```python
from build123d import *

# Parameters (mm, degrees)
LINK_PROFILE_SKETCH_R   = 7.5
LINK_PROFILE_SKETCH_R_2 = 20.85
LINK_BODY_15MM_DEPTH    = 15
BOLT_HOLE_SKETCH_R      = 5
BOLT_HOLE_10_DEPTH      = 159.633571478


with BuildPart() as part:
    # Link Profile Sketch → Link Body 15mm (new body)
    with BuildSketch(Plane.XY):
        with BuildLine():
            Line((100, 47), (92, 47))
            ThreePointArc((92, 47), (90.104459839, 21.32227727), (67.496938967, 9))
            Line((67.496938967, 9), (11.618950039, 9))
            ThreePointArc((11.618950039, 9), (6, 11.237900077), (0, 12))
            ThreePointArc((0, 12), (-12, 0), (0, -12))
            ThreePointArc((0, -12), (6, -11.237900077), (11.618950039, -9))
            Line((11.618950039, -9), (67.496938967, -9))
            ThreePointArc((67.496938967, -9), (90.104459839, -21.32227727), (92, -47))
            Line((92, -47), (100, -47))
            Line((100, -47), (108.73655718, -47))
            ThreePointArc((108.73655718, -47), (109.975380436, -32.246626192), (118.119137608, -19.882325124))
            ThreePointArc((118.119137608, -19.882325124), (126.899218543, 0.205040931), (117.813941305, 20.156227206))
            ThreePointArc((117.813941305, 20.156227206), (109.504751294, 32.334280207), (108, 47))
            Line((108, 47), (100, 47))
        make_face()
        Circle(LINK_PROFILE_SKETCH_R, mode=Mode.SUBTRACT)
        with Locations((100, 0)):
            Circle(LINK_PROFILE_SKETCH_R_2, mode=Mode.SUBTRACT)
        with BuildLine():
            Line((22.3, -5), (58.3, -5))
            ThreePointArc((58.3, -5), (63.3, 0), (58.3, 5))
            Line((58.3, 5), (22.3, 5))
            ThreePointArc((22.3, 5), (17.3, 0), (22.3, -5))
        make_face(mode=Mode.SUBTRACT)
    extrude(amount=LINK_BODY_15MM_DEPTH)

    # Bolt Hole Sketch → Bolt Hole Ø10 (cut, through all)
    with BuildSketch(Plane.XZ.offset(47)):
        with Locations(Location((100.36827859, 7.5, 0), (0, 0, 270))):
            Circle(BOLT_HOLE_SKETCH_R)
    extrude(amount=-BOLT_HOLE_10_DEPTH, mode=Mode.SUBTRACT)


solid = part.part
```
Read the model definition and answer for the solid it produces. Units are mm, in the model's axes. A direction names the side the tool comes from. Give positions to 0.01 mm unless a question says otherwise; leave off trailing zeros. Loops run counter-clockwise (first coordinate to the right, second up) from the corner with the lowest first, then second, coordinate; pieces in that order, holes last.
Item 1: The part is cut by section A-A (z = 8.5). Write down the section's boundary in (x, y).
Item 2: The part is cut by section B-B (y = 0). Write down the section's boundary in (x, z), and give its area (3 significant figures).
Item 3: For faces 4 (the flat face through (39, -9, 7)), 5 (the cylindrical face through (63.3, -0.1, 7.4)), 6 (the flat face through (40, 9, 7)), 7 (the flat face through (73, 0, 15)), determine the directions among +Z, -Z, +X, -X, +Y, -Y from which every point of the face is accessible in a straight line to the end or side of a thin tool.
Item 4: The part is cut by section C-C (x = 34.5). Write down the section's boundary in (y, z), and give its area (3 significant figures).
Item 5: Find the intervals of material crossed by line 1 along X through (y, z) = (-2, 3); line 2 along X through (y, z) = (-41.5, 9.25); line 3 along X through (y, z) = (29, 7.5), in increasing order.
Item 6: Each of these flat-tipped pins is pushed along its axis until it touches: pin 1 Ø6 at (x, z) = (66, 9.5) entering from +Y; pin 2 Ø5 at (y, z) = (11.5, 2.5) entering from -X; pin 3 Ø1.5 at (y, z) = (-35, 9) entering from -X. Where does it stop, or does it pass through?
Item 7: The mould has two halves that part along Y. Classify faces 1 (the flat face through (73, 0, 0)), 2 (the cylindrical face through (109.91, -32.44, 7.4)), 3 (the cylindrical face through (-12, 0, 7)): released by +Y, released by -Y, zero draft, split by the parting line, or undercut.
Item 8: The part is cut by section D-D (y = 34). Write down the section's boundary in (x, z), and give its area (3 significant figures).
Taken from the geometry:
1. outline: (0, -12) arc R24 ccw to (11.62, -9) - (67.5, -9) arc R26.9 cw to (92, -47) - (95.47, -47) - (95.47, -20.35) arc R20.85 cw to (95.47, 20.35) - (95.47, 47) - (92, 47) arc R26.9 cw to (67.5, 9) - (11.62, 9) arc R24 ccw to (0, 12) arc R12 ccw to start; (105.27, -47) - (108.74, -47) arc R30 cw to (118.12, -19.88) arc R26.9 ccw to (117.81, 20.16) arc R30 cw to (108, 47) - (105.27, 47) - (105.27, 20.17) arc R20.85 cw to (105.27, -20.17) - close; hole circle Ø15 at (0, 0); hole (22.3, -5) - (58.3, -5) arc R5 ccw to (58.3, 5) - (22.3, 5) arc R5 ccw to start
2. outline: (-12, 0) - (-7.5, 0) - (-7.5, 15) - (-12, 15) - close; (7.5, 0) - (17.3, 0) - (17.3, 15) - (7.5, 15) - close; (63.3, 0) - (79.15, 0) - (79.15, 15) - (63.3, 15) - close; (120.85, 0) - (126.9, 0) - (126.9, 15) - (120.85, 15) - close
2. area: 543 mm2
3. face 4: +Z, -Z, -Y
3. face 5: +Z, -Z
3. face 6: +Z, -Z, +Y
3. face 7: +Z, +X, -X, +Y, -Y
4. outline: (-9, 0) - (-5, 0) - (-5, 15) - (-9, 15) - close; (5, 0) - (9, 0) - (9, 15) - (5, 15) - close
4. area: 120 mm2
5. line 1: x = -11.83 to -7.23, 7.23 to 17.72, 62.88 to 79.25, 120.75 to 126.83
5. line 2: x = 93.81 to 95.68, 105.05 to 108.33
5. line 3: x = 93.5 to 95.37, 105.37 to 110.96
6. pin 1: stops at y = 9.04
6. pin 2: stops at x = -7.94
6. pin 3: stops at x = 94.35
7. face 1: zero draft
7. face 2: undercut
7. face 3: split by the parting line
8. outline: (94.33, 0) - (108.95, 0) - (108.95, 15) - (94.33, 15) - close; hole circle Ø10 at (100.37, 7.5)
8. area: 141 mm2
